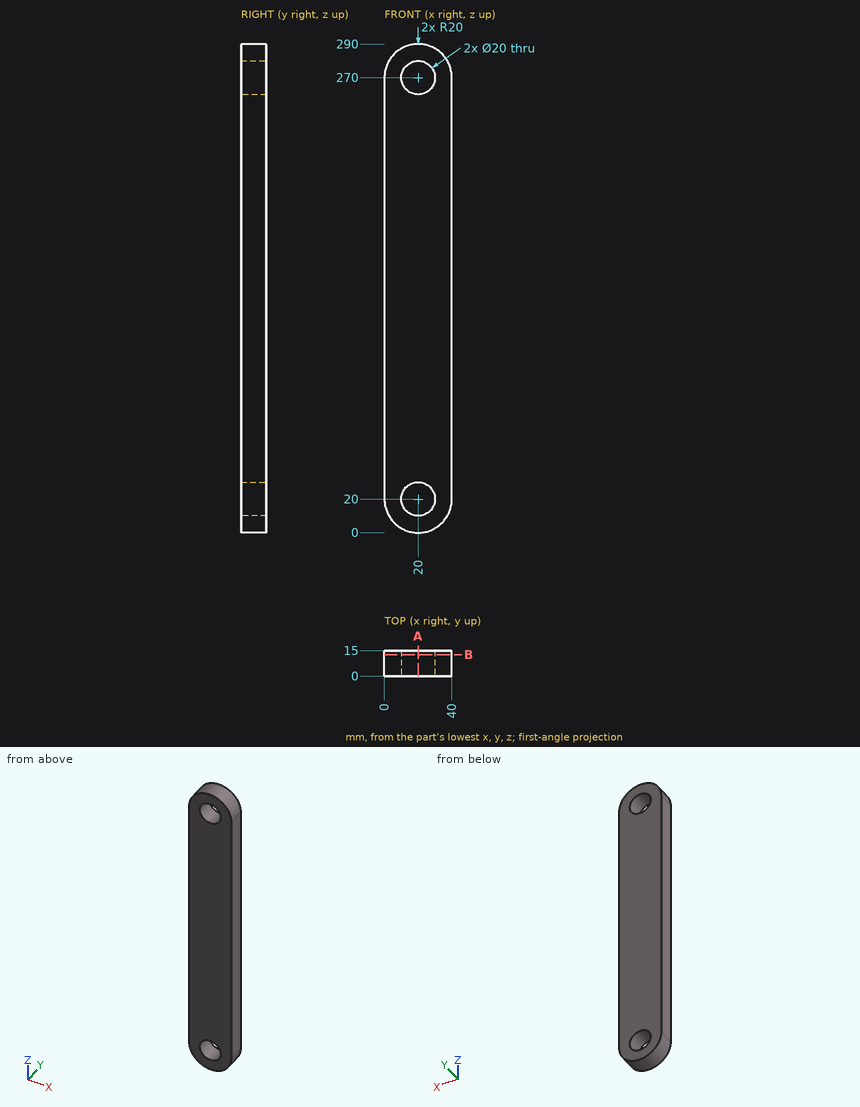
The figure shows three views and two pictorial views of one solid part (mm, origin at its lowest corner). Answer the questions. Give positions to 0.01 mm unless a question says otherwise; leave off trailing zeros. Order: outer loops, then holes, each group sorted by start corner. A loop starts at its lowest first (then second) coordinate and runs counter-clockwise, first axis right, second up. Notation, with made-up numbers: (77, 7) -> (93, 7) arc R20 cw to (93, 30) -> close; hole circle Ø2 at (63.25, 33). An arc over 180 degrees is marked (long way). Answer as CSV lines item,"result". Start each with the question number.
Q1. A cutting plane is placed at A-A (x = 20). Determine the outline of the cut face in (y, z), then the cut area to 3 significant figures.
Q2. Given pin 1 (3 mm diameter, centred on x = 16.5, y = 10, fed in from +Z); pin 2 (2 mm diameter, centred on x = 26.5, y = 1.5, fed in from -Z); pin 3 (2 mm diameter, centred on x = 34, y = 8.5, fed in from -Z), each flat-ended and moving along its own axis, determine where each tip first touches the part or whether it passes through.
Q3. A cutting plane is placed at B-B (y = 12.75). Determine the outline of the cut face in (x, z).
Q4. Find the intervals of material crossed by L1, parallel to Z at x = 23, y = 4; L2, parallel to Z at x = 16.5, y = 11; L3, parallel to X at y = 4, z = 20, in increasing order.
Results found:
1,outline,"(0, 0) -> (15, 0) -> (15, 10) -> (0, 10) -> close; (0, 30) -> (15, 30) -> (15, 260) -> (0, 260) -> close; (0, 280) -> (15, 280) -> (15, 290) -> (0, 290) -> close"
1,area,"3,750 mm2"
2,pin 1,"z = 289.9"
2,pin 2,"z = 0.77"
2,pin 3,"z = 4.8"
3,outline,"(0, 20) arc R20 ccw to (40, 20) -> (40, 270) arc R20 ccw to (0, 270) -> close; hole circle Ø20 at (20, 20); hole circle Ø20 at (20, 270)"
4,L1,"0.23 to 10.46, 29.54 to 260.46, 279.54 to 289.77"
4,L2,"0.31 to 10.63, 29.37 to 260.63, 279.37 to 289.69"
4,L3,"0 to 10, 30 to 40"
